from build123d import *

# Parameters (mm, degrees)
SKETCH1_W            = 615
SKETCH1_H            = 980
BOSS_EXTRUDE1_DEPTH  = 2
SKETCH7_W            = 45
SKETCH7_H            = 91
CUT_EXTRUDE4_DEPTH   = 579.498271389
SKETCH8_R            = 2.25
CUT_EXTRUDE5_DEPTH   = 579.498271389
FILLET3_R            = 10
CUT_EXTRUDE6_DEPTH   = 10
LPATTERN1_COUNT      = 3
LPATTERN1_PITCH      = 430
LPATTERN1_COUNT_DIR2 = 2
LPATTERN1_PITCH_DIR2 = 580


with BuildPart() as part:
    # Sketch1 → Boss-Extrude1 (new body)
    with BuildSketch(Plane.XY):
        Rectangle(SKETCH1_W, SKETCH1_H)
    extrude(amount=BOSS_EXTRUDE1_DEPTH)

    # Sketch7 → Cut-Extrude4 (cut, through all)
    with BuildSketch(Plane(origin=(0, 0, 0), x_dir=(-1, 0, 0), z_dir=(0, 0, -1))):
        with Locations((5, 300)):
            Rectangle(SKETCH7_W, SKETCH7_H)
        with Locations((5, -300)):
            Rectangle(SKETCH7_W, SKETCH7_H)
    extrude(amount=-CUT_EXTRUDE4_DEPTH, mode=Mode.SUBTRACT)

    # Sketch8 → Cut-Extrude5 (cut, through all)
    with BuildSketch(Plane(origin=(0, 0, 0), x_dir=(-1, 0, 0), z_dir=(0, 0, -1))):
        with Locations((5, 350)):
            Circle(SKETCH8_R)
        with Locations((5, 250)):
            Circle(SKETCH8_R)
        with Locations((5, -250)):
            Circle(SKETCH8_R)
        with Locations((5, -350)):
            Circle(SKETCH8_R)
    extrude(amount=-CUT_EXTRUDE5_DEPTH, mode=Mode.SUBTRACT)

    # Fillet3
    fillet3_edges = [part.edges().sort_by_distance(p)[0] for p in [
        (307.5, -490, 1),
        (-307.5, -490, 1),
        (-307.5, 490, 1),
        (307.5, 490, 1),
    ]]
    fillet(fillet3_edges, radius=FILLET3_R)

    # Sketch10 → Cut-Extrude6 (cut)
    with BuildSketch(Plane(origin=(0, 0, 0), x_dir=(-1, 0, 0), z_dir=(0, 0, -1))):
        with BuildLine():
            Line((292.5, 433.3), (286.9, 433.3))
            ThreePointArc((286.9, 433.3), (277, 430), (286.9, 426.7))
            Line((286.9, 426.7), (292.5, 426.7))
            ThreePointArc((292.5, 426.7), (295.8, 430), (292.5, 433.3))
        make_face()
    cut_extrude6 = extrude(amount=-CUT_EXTRUDE6_DEPTH, mode=Mode.SUBTRACT)

    # LPattern1: Cut-Extrude6 3 × 2
    with Locations(*[(j * LPATTERN1_PITCH_DIR2, -i * LPATTERN1_PITCH, 0) for i in range(LPATTERN1_COUNT) for j in range(LPATTERN1_COUNT_DIR2) if (i, j) != (0, 0)]):
        add(cut_extrude6, mode=Mode.SUBTRACT)


solid = part.part
Source: CAD feature listing. Evaluate the final solid. Frame: model axes, mm. Round coordinates to 2 decimals unless told otherwise and drop trailing zeros. Write item = value, one per line. Start each with the question number.
(1) Section query A-A, the plane z = 1.05. State how many separate pieces and enclosed holes the cut face has, plus the area to 3 significant figures.
(2) Pin query (flat end, axial travel): pin 1 (2.5 mm diameter, centred on x = -5, y = 350, fed in from -Z). Return the tip coordinate at first contact, or that it passes through.
(3) Ray query, line 1 along X through (y, z) = (430, 0.65); line 2 along Y through (x, z) = (297.5, 0.9); line 3 along Y through (x, z) = (-27, 1.15). Return the intervals inside material, ascending. Write a range as from..to.
Conclusion:
q1.separate_pieces = 1
q1.enclosed_holes = 12
q1.area = 593,000 mm2
q2.pin_1 = through
q3.line_1 = -307.5..-295.8, -277..284.2, 303..307.5
q3.line_2 = -490..-435.5, -424.5..-5.5, 5.5..424.5, 435.5..490
q3.line_3 = -490..-345.5, -254.5..254.5, 345.5..490
